Geometry check sheet. Reference: drawing and pictorial views, mm from the part's lowest x, y, z. A direction names the side the tool comes from. Give positions to 0.01 mm unless a question says otherwise; leave off trailing zeros. Write each loop counter-clockwise with the first axis right and the second up, starting at its lowest first coordinate (ties: lowest second). Pieces come first, ordered by that corner, then holes. Notation, with made-up numbers: (82, -34.75) - (129, -34.75) arc R31 cw to (129, -8.75) - close; hole circle Ø9 at (-34, 13.5). An arc over 180 degrees is marked (long way). Put each result on its own line as item: value.
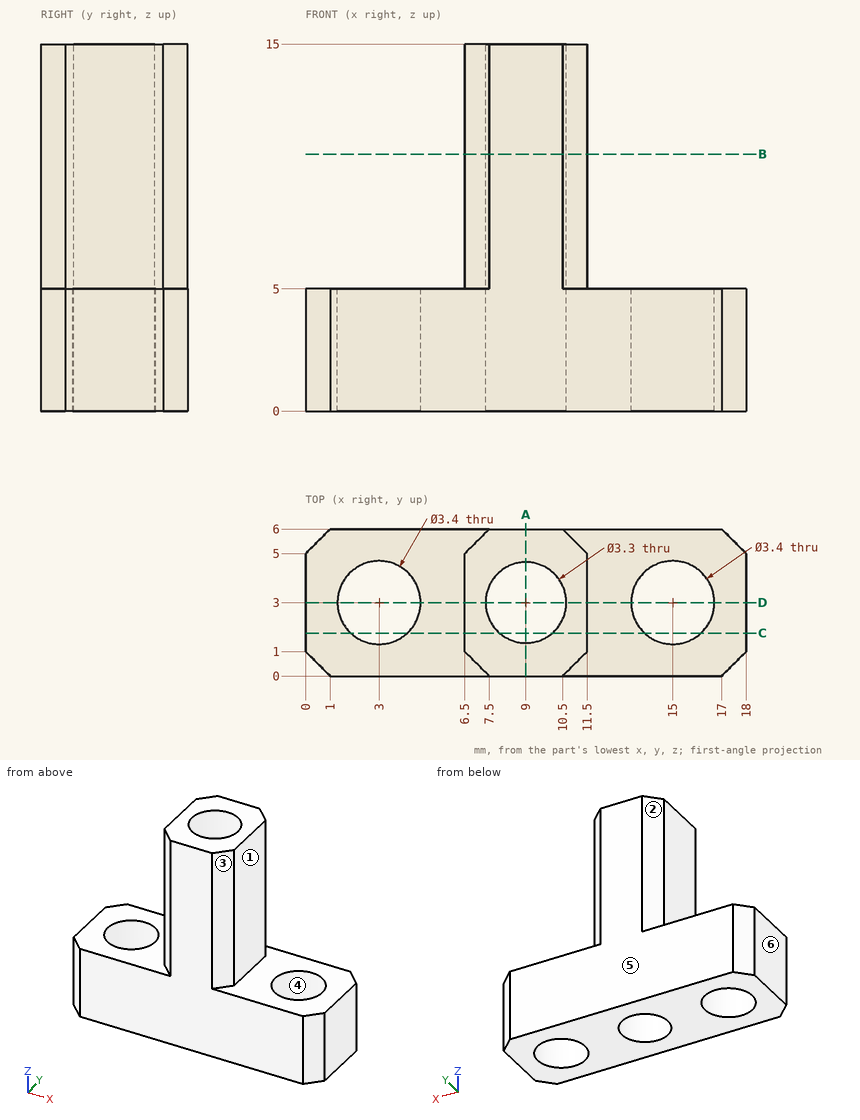
Q1. Go/stop test with flat-tipped pins: pin 1 Ø2.5 at (x, y) = (9, 3) entering from +Z; pin 2 Ø1.2 at (y, z) = (3, 9.5) entering from +X; pin 3 Ø1 at (y, z) = (3.5, 1.5) entering from -X; pin 4 Ø2 at (y, z) = (3.5, 7.5) entering from -X. Record where each tip stops, or that it passes through.
Answers follow:
pin 1: passes through
pin 2: stops at x = 11.5
pin 3: stops at x = 0
pin 4: stops at x = 6.5
Q2. Section check D-D, the plane y = 3. Record the cut outline in (x, z).
Answers follow:
outline: (0, 0) - (1.3, 0) - (1.3, 5) - (0, 5) - close; (4.7, 0) - (7.35, 0) - (7.35, 15) - (6.5, 15) - (6.5, 5) - (4.7, 5) - close; (10.65, 0) - (13.3, 0) - (13.3, 5) - (11.5, 5) - (11.5, 15) - (10.65, 15) - close; (16.7, 0) - (18, 0) - (18, 5) - (16.7, 5) - close
Q3. Scan lines: line 1 along Y through (x, z) = (15, 2.1); line 2 along X through (y, z) = (4.5, 2.25); line 3 along Z through (x, y) = (5.5, 5.5). Record each from-to range of solid material in increasing order.
Answers follow:
line 1: y = 0 to 1.3, 4.7 to 6
line 2: x = 0 to 2.2, 3.8 to 8.31, 9.69 to 14.2, 15.8 to 18
line 3: z = 0 to 5
Q4. Section check A-A, the plane x = 9. Record the cut outline in (y, z).
Answers follow:
outline: (0, 0) - (1.35, 0) - (1.35, 15) - (0, 15) - close; (4.65, 0) - (6, 0) - (6, 15) - (4.65, 15) - close
Q5. Release check for a two-part mould opening along Y. For the marked faces 4, 5 and 6 record: released by +Y, released by -Y, zero draft, split by the parting line, or undercut.
Answers follow:
face 4: undercut
face 5: released by +Y
face 6: zero draft
Q6. Section check B-B, the plane z = 10.5. Record the cut outline in (x, y), plus the area to 3 significant figures.
Answers follow:
outline: (6.5, 1) - (7.5, 0) - (10.5, 0) - (11.5, 1) - (11.5, 5) - (10.5, 6) - (7.5, 6) - (6.5, 5) - close; hole circle Ø3.3 at (9, 3)
area: 19.4 mm2
Q7. Set-up check for the marked faces 1, 2 and 3: record each of +Z, -Z, +X, -X, +Y, -Y from which the full face is reachable in a straight line by a thin tool's end or side.
Answers follow:
face 1: +Z, +X, +Y, -Y
face 2: +Z, -X, +Y
face 3: +Z, +X, -Y
Q8. Section check C-C, the plane y = 1.75. Record the cut outline in (x, z).
Answers follow:
outline: (0, 0) - (1.85, 0) - (1.85, 5) - (0, 5) - close; (4.15, 0) - (7.92, 0) - (7.92, 15) - (6.5, 15) - (6.5, 5) - (4.15, 5) - close; (10.08, 0) - (13.85, 0) - (13.85, 5) - (11.5, 5) - (11.5, 15) - (10.08, 15) - close; (16.15, 0) - (18, 0) - (18, 5) - (16.15, 5) - close
